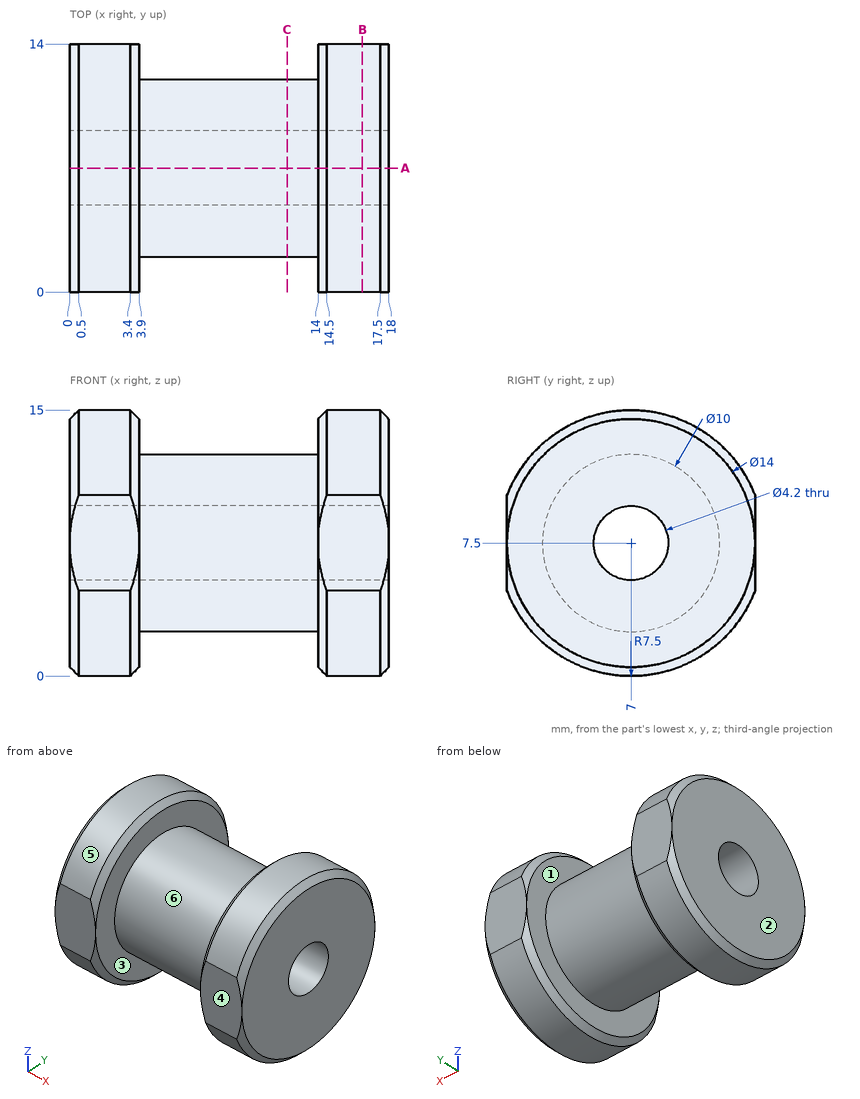
Source: three-view drawing plus pictorial views. Frame: mm from the lowest corner of the part. A direction names the side the tool comes from. Round coordinates to 2 decimals unless told otherwise and drop trailing zeros. Order: outer loops, then holes, each group sorted by start corner. A loop starts at its lowest first (then second) coordinate and runs counter-clockwise, first axis right, second up. Notation, with made-up numbers: (14.25, -10) -> (19.25, -10) arc R15 ccw to (19.25, 14) -> close; hole circle Ø3 at (62, 29). An arc over 180 degrees is marked (long way). Use one line per item in the form item = value. Start each with the question number.
1. Pin query (flat end, axial travel): pin 1 Ø1.5 at (y, z) = (7.5, 11) entering from -X; pin 2 Ø6 at (x, z) = (9, 8.5) entering from -Y; pin 3 Ø8 at (x, y) = (9.5, 7.5) entering from +Z. Return the tip coordinate at first contact, or that it passes through.
2. Cut plane C-C (x = 12.25). Return the cut outline in (y, z).
3. Cut plane A-A (y = 7). Return the cut outline in (x, z).
4. Draft query along X for the marked faces 1, 2, 3 and 4. Return one class per face: pulls with the +X half, pulls with the -X half, needs draft (parallel to the pull), parting line crosses it, or undercut.
5. Line query: probe 1 along X at (y, z) = (1.75, 8); probe 2 along Y at (x, z) = (4, 7.5); probe 3 along Z at (x, y) = (16.5, 8.75). Output: solid intervals per line, ascending.
6. Cut plane B-B (x = 16.5). Return the cut outline in (y, z), then the cut area to 3 significant figures.
7. Reachability of the marked faces 5 and 6 from +Z, -Z, +X, -X, +Y, -Y: full face, straight path, thin tool, end or side. Return the list, or none.
Solution:
q1.pin_1 = 0
q1.pin_2 = 2
q1.pin_3 = 12.5
q2.outline = circle Ø10 at (7, 7.5); hole circle Ø4.2 at (7, 7.5)
q3.outline = (0, 0.5) -> (0.5, 0) -> (3.4, 0) -> (3.9, 0.5) -> (3.9, 2.5) -> (14, 2.5) -> (14, 0.5) -> (14.5, 0) -> (17.5, 0) -> (18, 0.5) -> (18, 5.4) -> (0, 5.4) -> close; (0, 9.6) -> (18, 9.6) -> (18, 14.5) -> (17.5, 15) -> (14.5, 15) -> (14, 14.5) -> (14, 12.5) -> (3.9, 12.5) -> (3.9, 14.5) -> (3.4, 15) -> (0.5, 15) -> (0, 14.5) -> close
q4.face_1 = undercut
q4.face_2 = pulls with the -X half
q4.face_3 = undercut
q4.face_4 = needs draft
q5.probe_1 = 0 to 3.9, 14 to 18
q5.probe_2 = 2 to 4.9, 9.1 to 12
q5.probe_3 = 0.21 to 6.34, 8.66 to 14.79
q6.outline = (0, 4.81) arc R7.5 ccw to (14, 4.81) -> (14, 10.19) arc R7.5 ccw to (0, 10.19) -> close; hole circle Ø4.2 at (7, 7.5)
q6.area = 159 mm^2
q7.face_5 = +Z, +X, -X
q7.face_6 = none
